The listing builds one solid part. Answer for the finished solid, in the listing's coordinates (mm). A direction names the side the tool comes from. Round coordinates to 2 decimals unless told otherwise and drop trailing zeros. Loops run counter-clockwise (first coordinate to the right, second up) from the corner with the lowest first, then second, coordinate; pieces in that order, holes last. Notation, with made-up numbers: (20.5, -17.5) - (78.5, -17.5) arc R30 cw to (78.5, 19.5) - close; hole circle Ø8 at (81, -15.75). An arc over 180 degrees is marked (long way). Write item = value, one per line. Start each with the question number.
1) Section D-D, the plane y = 15.5 is taken. Determine the outline of the cut face in (x, z).
2) A tool of negligible diameter and unlimited length cuts with its end or side. For faces 4 (the cylindrical face through (12.394, -0.378, 1.627)), 5 (the flat face through (-27, -10.2, 0.1)), from which of +Z, -Z, +X, -X, +Y, -Y can it reach the whole face along a straight path? Write none if from no direction.
3) Section B-B, the plane x = 4 is taken. Determine the outline of the cut face in (y, z), and give its area (3 significant figures).
4) For a pull along Z with two mould halves and no side action, classify faces 1 (the cylindrical face through (9.915, -0.378, 1.302)), 2 (the flat face through (-10.2, 27, 0.1)), 3 (the cylindrical face through (-16.69, -8.45, 9.21)) as released by +Z, released by -Z, zero draft, split by the parting line, or undercut.
5) Section C-C, the plane y = 0 is taken. Determine the outline of the cut face in (x, z), and give its area (3 significant figures).
6) Section A-A, the plane z = 0 is taken. Determine the outline of the cut face in (x, y), and give its area (4 significant figures).
7) Straight lines are drawn through the part: line 1 along Y through (x, z) = (-16.5, 0); line 2 along X through (y, z) = (10, 2). For each, find the intervals that lie inside material, in ascending order.
8) Given pin 1 Ø5 at (x, y) = (-18.5, -8) entering from -Z (3 decimals); pin 2 Ø10 at (y, z) = (2, 2) entering from -X; pin 3 Ø8 at (y, z) = (-13.5, 8.5) entering from +X; pin 4 Ø6 at (x, z) = (-14, 5) entering from +Y, each flat-ended and moving along its own axis, determine where each tip first touches the part or whether it passes through.
from build123d import *

# Parameters (mm, degrees)
SKETCH_1_W               = 2.5
SKETCH_1_H               = 27
PATTERN_CIRCULAR_1_COUNT = 3
PATTERN_CIRCULAR_1_ANGLE = 180
SKETCH_2_R               = 10
CUT_EXTRUDE_1_DEPTH      = 62.654278166
SKETCH_3_R               = 10
CUT_EXTRUDE_2_DEPTH      = 41.177730217


with BuildPart() as part:
    # 草图1 → 旋转1 (revolve)
    with BuildSketch(Plane.XY, mode=Mode.PRIVATE) as revolve_1_sk:
        with Locations((-11.25, 13.5)):
            Rectangle(SKETCH_1_W, SKETCH_1_H)
    revolve_1 = revolve(revolve_1_sk.sketch.rotate(Axis((0, 0, 0), (0, 1, 0)), 270), axis=Axis((0, 0, 0), (0, 1, 0)))

    # 阵列(圆周)1: 旋转1 ×3 about axis
    pattern_circular_1_axis = Axis((0, 0, 0), (0, 0, 1))
    for i in range(1, PATTERN_CIRCULAR_1_COUNT):
        add(revolve_1.rotate(pattern_circular_1_axis, i * PATTERN_CIRCULAR_1_ANGLE / (PATTERN_CIRCULAR_1_COUNT - 1)))

    # 草图2 → 切除-拉伸1 (cut, through all)
    with BuildSketch(Plane.XZ.offset(27)):
        with Locations(Location((0, 0, 0), (0, 0, 270))):
            Circle(SKETCH_2_R)
    extrude(amount=-CUT_EXTRUDE_1_DEPTH, mode=Mode.SUBTRACT)

    # 草图3 → 切除-拉伸2 (cut, through all)
    with BuildSketch(Plane(origin=(0, 0, 0), x_dir=(0, 0, -1), z_dir=(1, 0, 0))):
        Circle(SKETCH_3_R)
    extrude(amount=-CUT_EXTRUDE_2_DEPTH, mode=Mode.SUBTRACT)


solid = part.part
Geometry check:
q1.outline = circle Ø25 at (0, 0); hole circle Ø20 at (0, 0)
q2.face_4 = none
q2.face_5 = +Z, -Z, -X, +Y, -Y
q3.outline = (-27, -11.84) - (27, -11.84) - (27, -9.17) - (-27, -9.17) - close; (-27, 9.17) - (27, 9.17) - (27, 11.84) - (-27, 11.84) - close
q3.area = 289 mm2
q4.face_1 = undercut
q4.face_2 = zero draft
q4.face_3 = split by the parting line
q5.outline = (-27, -12.5) - (0, -12.5) arc R12.5 ccw to (0, 12.5) - (-27, 12.5) - (-27, 10) - (0, 10) arc R10 cw to (0, -10) - (-27, -10) - close
q5.area = 223 mm2
q6.outline = (-27, -12.5) - (-12.5, -12.5) - (-12.5, -27) - (-10, -27) - (-10, -10) - (-27, -10) - close; (-27, 10) - (-10, 10) - (-10, 27) - (-12.5, 27) - (-12.5, 12.5) - (-27, 12.5) - close; (10, -27) - (12.5, -27) - (12.5, 27) - (10, 27) - close
q6.area = 292.5 mm2
q7.line_1 = -12.5 to -10, 10 to 12.5
q7.line_2 = -27 to -9.8, 9.8 to 12.34
q8.pin_1 = -11.225
q8.pin_2 = 7.14
q8.pin_3 = 11.66
q8.pin_4 = 27
